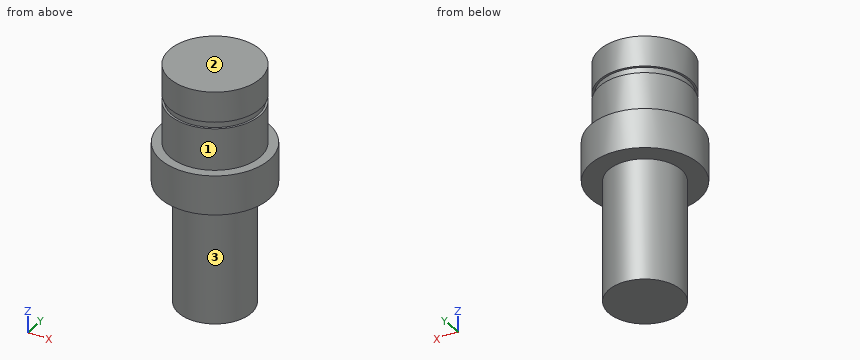
from build123d import *

# Parameters (mm, degrees)
CUT_EXTRUDE_START   = -1.1
SKETCH_3_R          = 7.5
SKETCH_3_R_2        = 7.15
CUT_EXTRUDE_1_DEPTH = 1.1


with BuildPart() as part:
    # 草图2 → 旋转1 (revolve)
    with BuildSketch(Plane(origin=(0, 0, 0), x_dir=(0, 0, -1), z_dir=(1, 0, 0)), mode=Mode.PRIVATE) as revolve_1_sk:
        Polygon((0, 0), (0, 7.5), (13, 7.5), (13, 9), (19.5, 9), (19.5, 6), (39.5, 6), (39.5, 0), align=None)
    revolve(revolve_1_sk.sketch.rotate(Axis((0, 0, -39.5), (0, 0, 1)), 90), axis=Axis((0, 0, -39.5), (0, 0, 1)))

    # 草图3 → 切除-拉伸1 (cut)
    with BuildSketch(Plane.XY.offset(-5).offset(CUT_EXTRUDE_START)):
        with Locations(Location((0, 0, 0), (0, 0, 180))):
            Circle(SKETCH_3_R)
        Circle(SKETCH_3_R_2, mode=Mode.SUBTRACT)
    extrude(amount=CUT_EXTRUDE_1_DEPTH, mode=Mode.SUBTRACT)


solid = part.part
Input: part model. Units: mm. Frame: model coordinates. Face numbers are marked on the shaded views. A direction names the side the tool comes from. Give positions to 0.01 mm unless a question says otherwise; leave off trailing zeros. Write each loop counter-clockwise with the first axis right and the second up, starting at its lowest first coordinate (ties: lowest second). Pieces come first, ordered by that corner, then holes. Notation, with made-up numbers: (20.25, -17) -> (32.25, -17) arc R36 ccw to (32.25, 17) -> close; hole circle Ø5 at (71.5, -6.5). An arc over 180 degrees is marked (long way). Use one line per item in the form item = value. Start each with the question number.
1) Section query C-C on z = -14. Return the cut outline in (x, y), then the cut area to 3 significant figures.
2) Section query D-D on y = 6.5. Return the cut outline in (x, z).
3) Pin query (flat end, axial travel): pin 1 (5 mm diameter, centred on y = 7, z = -29.5, fed in from +X); pin 2 (5 mm diameter, centred on x = 5, z = -29, fed in from +Y); pin 3 (5 mm diameter, centred on y = -1.5, z = -9.5, fed in from -X). Return the tip coordinate at first contact, or that it passes through.
4) Ray query, probe 1 along Z at (x, y) = (-7.25, 1.5); probe 2 along Z at (x, y) = (-3.5, -6); probe 3 along Z at (x, y) = (-5.5, 5.5). Return the intervals inside material, ascending. Write a range as from..to.
5) Set-up query: the marked faces 1, 2 and 3. Return all of +Z, -Z, +X, -X, +Y, -Y with unobstructed straight access to the full face (end or side cutting, diameter ignored); none if empty.
6) Section query A-A on y = 0. Return the cut outline in (x, z).
Outcome:
q1.outline = circle Ø18 at (0, 0)
q1.area = 254 mm^2
q2.outline = (-6.22, -19.5) -> (6.22, -19.5) -> (6.22, -13) -> (3.74, -13) -> (3.74, -6.1) -> (2.98, -6.1) -> (2.98, -5) -> (3.74, -5) -> (3.74, 0) -> (-3.74, 0) -> (-3.74, -5) -> (-2.98, -5) -> (-2.98, -6.1) -> (-3.74, -6.1) -> (-3.74, -13) -> (-6.22, -13) -> close
q3.pin_1 = 3.97
q3.pin_2 = 5.45
q3.pin_3 = -7.5
q4.probe_1 = -19.5..-6.1, -5..0
q4.probe_2 = -19.5..0
q4.probe_3 = -19.5..-13
q5.face_1 = +Z
q5.face_2 = +Z, +X, -X, +Y, -Y
q5.face_3 = -Z
q6.outline = (-9, -19.5) -> (-6, -19.5) -> (-6, -39.5) -> (6, -39.5) -> (6, -19.5) -> (9, -19.5) -> (9, -13) -> (7.5, -13) -> (7.5, -6.1) -> (7.15, -6.1) -> (7.15, -5) -> (7.5, -5) -> (7.5, 0) -> (-7.5, 0) -> (-7.5, -5) -> (-7.15, -5) -> (-7.15, -6.1) -> (-7.5, -6.1) -> (-7.5, -13) -> (-9, -13) -> close
